Could you check a few things on this drawing? It's one solid part, dimensions in mm from its lowest x, y, z. Coordinates: 2 decimals unless noted, no trailing zeros. Loops run counter-clockwise (first coordinate to the right, second up) from the corner with the lowest first, then second, coordinate; pieces in that order, holes last. Notation, with made-up numbers: (41.25, -22) -> (100.25, -22) arc R8 cw to (100.25, -15) -> close; hole circle Ø10 at (-13.5, -20). An arc over 180 degrees is marked (long way). One line per question, with ' | ' between items. Start each with the question number.
(1) Suppose I cut it at B-B (x = 4). Please give me the cut outline in (y, z), plus the area to 3 significant figures.
(2) Suppose I cut it at A-A (y = 4). Please give me the cut outline in (x, z), plus the area to 3 significant figures.
(3) Suppose I cut it at D-D (x = 21). Please give me the cut outline in (y, z), plus the area to 3 significant figures.
(4) If I drill on line 1 along Y through (x, z) = (4, 0.2); line 2 along X through (y, z) = (3, 0.45); line 3 along X through (y, z) = (4.75, 0.4), over which ranges is the centre line in solid material (lowest first)?
(5) I'm going to push flat-ended pins straight in: pin 1 Ø4 at (x, y) = (22.5, 5) entering from -Z; pin 2 Ø2.5 at (x, y) = (4, 4) entering from +Z (1 decimal). Where does each tip first touch, or does it pass through?
(6) Suppose I cut it at C-C (z = 0.65). Please give me the cut outline in (x, y).
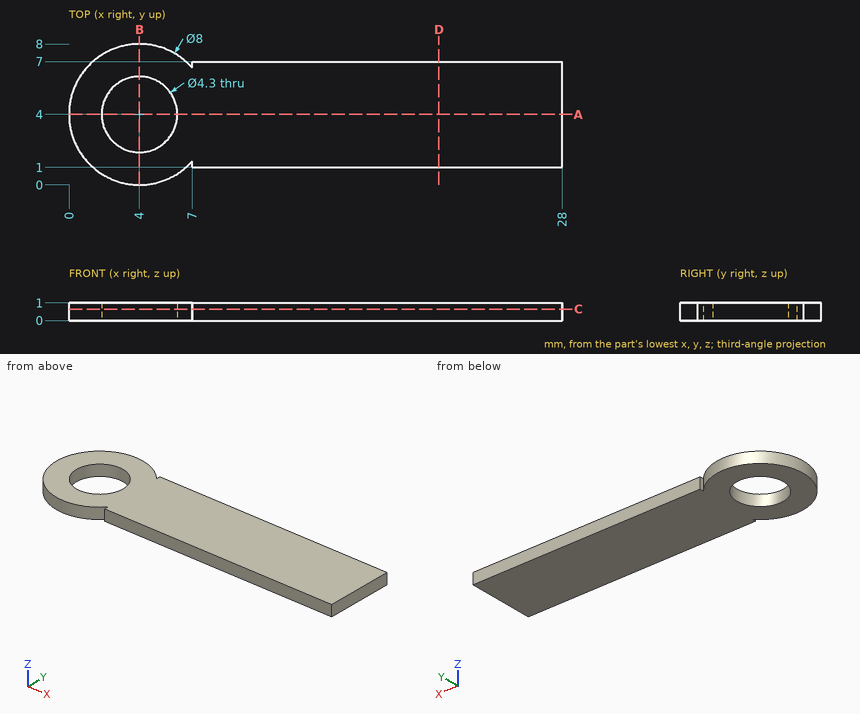
Checks:
1) outline: (0, 0) -> (1.85, 0) -> (1.85, 1) -> (0, 1) -> close; (6.15, 0) -> (8, 0) -> (8, 1) -> (6.15, 1) -> close | area: 3.70 mm^2
2) outline: (0, 0) -> (1.85, 0) -> (1.85, 1) -> (0, 1) -> close; (6.15, 0) -> (28, 0) -> (28, 1) -> (6.15, 1) -> close | area: 23.7 mm^2
3) outline: (1, 0) -> (7, 0) -> (7, 1) -> (1, 1) -> close | area: 6.00 mm^2
4) line 1: y = 0 to 1.85, 6.15 to 8 | line 2: x = 0.13 to 2.1, 5.9 to 28 | line 3: x = 0.07 to 1.99, 6.01 to 28
5) pin 1: stops at z = 0 | pin 2: passes through
6) outline: (7, 1) -> (28, 1) -> (28, 7) -> (7, 7) -> (7, 6.65) arc R4 ccw (long way) to (7, 1.35) -> close; hole circle Ø4.3 at (4, 4)
